```python
from build123d import *

# Parameters (mm, degrees)
BASE_PLATE_SKETCH_W                    = 15
BASE_PLATE_SKETCH_H                    = 8
BASE_PLATE_15X8X2_DEPTH                = 2
HIP_BLOCKS_SKETCH_W                    = 3.8
HIP_BLOCKS_SKETCH_H                    = 3.6
HIP_BLOCKS_DRAFTED_5MM_DEPTH           = 5
HIP_BLOCKS_DRAFTED_5MM_DRAFT           = 7
HIP_BLOCKS_DRAFTED_5MM_PROFILE_2_DEPTH = 5
HIP_BLOCKS_DRAFTED_5MM_PROFILE_2_DRAFT = 7
UNDERSIDE_RELIEF_SKETCH_R              = 4
UNDERSIDE_RELIEF_CUT_DEPTH             = 19.384776311
HIP_DISC_SKETCH_R                      = 4
HIP_DISC_8_DEPTH                       = 1
AXLE_PIN_A_SKETCH_R                    = 1.5
AXLE_PIN_A_3_DEPTH                     = 1
AXLE_PIN_B_SKETCH_R                    = 1.5
AXLE_PIN_B_3_DEPTH                     = 1


with BuildPart() as part:
    # Base Plate Sketch → Base Plate 15x8x2 (new body)
    with BuildSketch(Plane(origin=(0, 0, 0), x_dir=(1, 0, 0), z_dir=(0, 1, 0))):
        with Locations((7.5, 4)):
            Rectangle(BASE_PLATE_SKETCH_W, BASE_PLATE_SKETCH_H)
    extrude(amount=BASE_PLATE_15X8X2_DEPTH)


with BuildPart() as hip_blocks_drafted_5mm_tool:
    # Hip Blocks Sketch → Hip Blocks Drafted 5mm (with draft: the straight prism first)
    with BuildSketch(Plane(origin=(0, 2, 0), x_dir=(1, 0, 0), z_dir=(0, 1, 0))):
        with Locations((4.1, 4)):
            Rectangle(HIP_BLOCKS_SKETCH_W, HIP_BLOCKS_SKETCH_H)
    extrude(amount=HIP_BLOCKS_DRAFTED_5MM_DEPTH)
    # Hip Blocks Drafted 5mm: the draft: its side faces are tilted about the plane it starts from
    hip_blocks_drafted_5mm_sides = [hip_blocks_drafted_5mm_tool.faces().sort_by_distance(p)[0] for p in [
        (2.2, 4.5, -4),
        (4.1, 4.5, -2.2),
        (6, 4.5, -4),
        (4.1, 4.5, -5.8),
    ]]
    draft(hip_blocks_drafted_5mm_sides, Plane(origin=(0, 2, 0), x_dir=(1, 0, 0), z_dir=(0, 1, 0)), HIP_BLOCKS_DRAFTED_5MM_DRAFT)


with BuildPart() as part_1:
    add(part.part)

    # Hip Blocks Drafted 5mm: add hip_blocks_drafted_5mm_tool
    add(hip_blocks_drafted_5mm_tool.part)


with BuildPart() as hip_blocks_drafted_5mm_profile_2_tool:
    # Hip Blocks Sketch → Hip Blocks Drafted 5mm profile 2 (with draft: the straight prism first)
    with BuildSketch(Plane(origin=(0, 2, 0), x_dir=(1, 0, 0), z_dir=(0, 1, 0))):
        with Locations((10.9, 4)):
            Rectangle(HIP_BLOCKS_SKETCH_W, HIP_BLOCKS_SKETCH_H)
    extrude(amount=HIP_BLOCKS_DRAFTED_5MM_PROFILE_2_DEPTH)
    # Hip Blocks Drafted 5mm profile 2: the draft: its side faces are tilted about the plane it starts from
    hip_blocks_drafted_5mm_profile_2_sides = [hip_blocks_drafted_5mm_profile_2_tool.faces().sort_by_distance(p)[0] for p in [
        (10.9, 4.5, -5.8),
        (9, 4.5, -4),
        (10.9, 4.5, -2.2),
        (12.8, 4.5, -4),
    ]]
    draft(hip_blocks_drafted_5mm_profile_2_sides, Plane(origin=(0, 2, 0), x_dir=(1, 0, 0), z_dir=(0, 1, 0)), HIP_BLOCKS_DRAFTED_5MM_PROFILE_2_DRAFT)


with BuildPart() as part_2:
    add(part_1.part)

    # Hip Blocks Drafted 5mm profile 2: add hip_blocks_drafted_5mm_profile_2_tool
    add(hip_blocks_drafted_5mm_profile_2_tool.part)

    # Underside Relief Sketch → Underside Relief Cut (cut, through all)
    with BuildSketch(Plane(origin=(15, 0, 0), x_dir=(0, 0, -1), z_dir=(1, 0, 0))):
        with Locations((4, -2.5)):
            Circle(UNDERSIDE_RELIEF_SKETCH_R)
    extrude(amount=-UNDERSIDE_RELIEF_CUT_DEPTH, mode=Mode.SUBTRACT)

    # Hip Disc Sketch → Hip Disc Ø8 (add, symmetric)
    with BuildSketch(Plane.ZY.offset(-7.5)):
        with Locations((-4, -2.5)):
            Circle(HIP_DISC_SKETCH_R)
    extrude(amount=HIP_DISC_8_DEPTH, both=True)

    # Axle Pin A Sketch → Axle Pin A Ø3 (add, symmetric)
    with BuildSketch(Plane(origin=(8.5, 0, 0), x_dir=(0, 0, -1), z_dir=(1, 0, 0))):
        with Locations(Location((4, -2.5, 0), (0, 0, 180))):
            Circle(AXLE_PIN_A_SKETCH_R)
    extrude(amount=AXLE_PIN_A_3_DEPTH, both=True)

    # Axle Pin B Sketch → Axle Pin B Ø3 (add, symmetric)
    with BuildSketch(Plane.ZY.offset(-6.5)):
        with Locations((-4, -2.5)):
            Circle(AXLE_PIN_B_SKETCH_R)
    extrude(amount=AXLE_PIN_B_3_DEPTH, both=True)


solid = part_2.part
```
Source: CAD feature listing. Evaluate the final solid. Frame: model axes, mm. A direction names the side the tool comes from. Give positions to 0.01 mm unless a question says otherwise; leave off trailing zeros. Write each loop counter-clockwise with the first axis right and the second up, starting at its lowest first coordinate (ties: lowest second). Pieces come first, ordered by that corner, then holes. Notation, with made-up numbers: (42, 56) - (47, 56) arc R20 ccw to (47, 80) - close; hole circle Ø7 at (31.25, 79.5). An arc over 180 degrees is marked (long way). One line per item, written item: value. Start each with the question number.
Q1. Section query C-C, the plane y = -2.5. Return the cut outline in (x, z).
Q2. Section query D-D, the plane z = -4. Return the cut outline in (x, y), then the cut area to 3 significant figures.
Q3. Section query B-B, the plane x = 10. Return the cut outline in (y, z), then the cut area to 3 significant figures.
Q4. First-contact query: pin 1 Ø2.5 at (y, z) = (-4, -3) entering from +X; pin 2 Ø4 at (y, z) = (-1, -5) entering from -X; pin 3 Ø1 at (x, z) = (5, -7.5) entering from -Y. Flat tips, straight axial feed; report the tip coordinate or a pass-through.
Q5. Set-up query: faces 4 (the face through (5.5, -2, -4)), 5 (the face through (9.5, -3, -4)), 6 (the face through (6.5, -2, -2)), 7 (the face through (9.303, 4.465, -3.975)). Return all of +Z, -Z, +X, -X, +Y, -Y with unobstructed straight access to the full face (end or side cutting, diameter ignored); none if empty.
Q6. Draft query along Y for faces 1 (the face through (2.503, 4.465, -3.975)), 2 (the face through (7, 1, -8)), 3 (the face through (5.993, -1.235, -3.194)). Return one class per face: +Y half, -Y half, draft (parallel to the pull), parting line (faces both ways), or undercut.
Q7. Material intervals for probe 1 along X at (y, z) = (-4.75, -3.5); probe 2 along Y at (x, z) = (11.5, -0.25); probe 3 along X at (y, z) = (3.25, -2.5), sorted ascending. Write a range as from..to.
Q8. Section query A-A, the plane y = 2.5. Return the cut outline in (x, z), then the cut area to 3 significant figures.
Answer:
1. outline: (5.5, -5.5) - (6.5, -5.5) - (6.5, -8) - (8.5, -8) - (8.5, -5.5) - (9.5, -5.5) - (9.5, -2.5) - (8.5, -2.5) - (8.5, 0) - (6.5, 0) - (6.5, -2.5) - (5.5, -2.5) - close
2. outline: (0, 1.5) - (6.5, 1.5) - (6.5, -1) - (5.5, -1) - (5.5, -4) - (6.5, -4) - (6.5, -6.5) - (8.5, -6.5) - (8.5, -4) - (9.5, -4) - (9.5, -1) - (8.5, -1) - (8.5, 1.5) - (15, 1.5) - (15, 2) - (12.8, 2) - (12.19, 7) - (9.61, 7) - (9, 2) - (6, 2) - (5.39, 7) - (2.81, 7) - (2.2, 2) - (0, 2) - close
2. area: 61.4 mm2
3. outline: (0, -8) - (2, -8) - (2, -5.8) - (7, -5.19) - (7, -2.81) - (2, -2.2) - (2, 0) - (0, 0) - (0, -0.88) arc R4 cw to (0, -7.12) - close
3. area: 24.4 mm2
4. pin 1: stops at x = 9.5
4. pin 2: stops at x = 5.5
4. pin 3: stops at y = 0
5. face 4: +Z, -Z, -X, -Y
5. face 5: +Z, -Z, +X, -Y
5. face 6: -X
5. face 7: +Z, -Z, +Y
6. face 1: +Y half
6. face 2: draft
6. face 3: undercut
7. probe 1: x = 6.5..8.5
7. probe 2: y = 0..2
7. probe 3: x = 2.35..5.85, 9.15..12.65
8. outline: (2.26, -5.74) - (5.94, -5.74) - (5.94, -2.26) - (2.26, -2.26) - close; (9.06, -5.74) - (12.74, -5.74) - (12.74, -2.26) - (9.06, -2.26) - close
8. area: 25.6 mm2
